For this review, take the finished solid that the model builds, in its own axes (mm). Face numbers are marked on the shaded views. A direction names the side the tool comes from. Round coordinates to 2 decimals unless told otherwise and drop trailing zeros. Write each loop counter-clockwise with the first axis right and the second up, starting at its lowest first coordinate (ties: lowest second). Pieces come first, ordered by that corner, then holes. Notation, with made-up numbers: M -5.5,52.5 L 43.5,52.5 A11 ccw 43.5,68.5 Z; hole C -13.5,33.25 d10. An arc over 180 degrees is marked long. Answer in a Markdown table with one row per item.
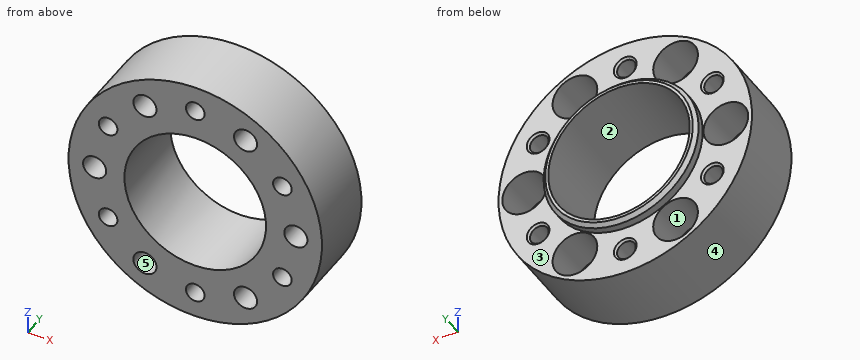
```python
from build123d import *

# Parameters (mm, degrees)
SKETCH_1_R                   = 17
SKETCH_1_R_2                 = 1.55
SKETCH_1_R_3                 = 9.5
EXTRUDE_1_DEPTH              = 9.5
HOLE_WIZARD_M3_1_D           = 2.5
HOLE_WIZARD_M3_1_CSINK_D     = 3.05
HOLE_WIZARD_M3_1_CSINK_ANGLE = 90
SKETCH_7_R                   = 10.4
SKETCH_7_R_2                 = 9.5
EXTRUDE_2_DEPTH              = 1.5
SKETCH_5_R                   = 3
CUT_EXTRUDE_1_DEPTH          = 5.5
CHAMFER_1_SIZE               = 0.5


with BuildPart() as part:
    # 草图1 → 凸台-拉伸1 (new body)
    with BuildSketch(Plane(origin=(0, 0, 0), x_dir=(1, 0, 0), z_dir=(0, 1, 0))):
        with Locations(Location((0, 0, 0), (0, 0, 270))):
            Circle(SKETCH_1_R)
        with Locations(Location((13.5, 0, 0), (0, 0, 270))):
            Circle(SKETCH_1_R_2, mode=Mode.SUBTRACT)
        with Locations(Location((6.75, -11.691342951, 0), (0, 0, 270))):
            Circle(SKETCH_1_R_2, mode=Mode.SUBTRACT)
        with Locations(Location((-6.75, -11.691342951, 0), (0, 0, 270))):
            Circle(SKETCH_1_R_2, mode=Mode.SUBTRACT)
        with Locations(Location((-13.5, 0, 0), (0, 0, 270))):
            Circle(SKETCH_1_R_2, mode=Mode.SUBTRACT)
        with Locations(Location((-6.75, 11.691342951, 0), (0, 0, 270))):
            Circle(SKETCH_1_R_2, mode=Mode.SUBTRACT)
        with Locations(Location((6.75, 11.691342951, 0), (0, 0, 270))):
            Circle(SKETCH_1_R_2, mode=Mode.SUBTRACT)
        with Locations(Location((0, 0, 0), (0, 0, 270))):
            Circle(SKETCH_1_R_3, mode=Mode.SUBTRACT)
    extrude(amount=EXTRUDE_1_DEPTH)

    # M3 螺纹孔1 (through all)
    with Locations(Plane(origin=(0, 9.5, 0), x_dir=(1, 0, 0), z_dir=(0, 1, 0))):
        with Locations((11.691342951, 6.75), (11.691342951, -6.75), (0, -13.5), (-11.691342951, -6.75), (-11.691342951, 6.75), (0, 13.5), (0, 0)):
            CounterSinkHole(HOLE_WIZARD_M3_1_D / 2, HOLE_WIZARD_M3_1_CSINK_D / 2, counter_sink_angle=HOLE_WIZARD_M3_1_CSINK_ANGLE)

    # 草图7 → 凸台-拉伸2 (add)
    with BuildSketch(Plane(origin=(0, 9.5, 0), x_dir=(1, 0, 0), z_dir=(0, 1, 0))):
        with Locations(Location((0, 0, 0), (0, 0, 270))):
            Circle(SKETCH_7_R)
        with Locations(Location((0, 0, 0), (0, 0, 270))):
            Circle(SKETCH_7_R_2, mode=Mode.SUBTRACT)
    extrude(amount=EXTRUDE_2_DEPTH)

    # 草图5 → 切除-拉伸1 (cut)
    with BuildSketch(Plane(origin=(0, 9.5, 0), x_dir=(1, 0, 0), z_dir=(0, 1, 0))):
        with Locations(Location((13.5, 0, 0), (0, 0, 270))):
            Circle(SKETCH_5_R)
        with Locations(Location((6.75, -11.691342951, 0), (0, 0, 270))):
            Circle(SKETCH_5_R)
        with Locations(Location((-6.75, -11.691342951, 0), (0, 0, 270))):
            Circle(SKETCH_5_R)
        with Locations(Location((-13.5, 0, 0), (0, 0, 270))):
            Circle(SKETCH_5_R)
        with Locations(Location((-6.75, 11.691342951, 0), (0, 0, 270))):
            Circle(SKETCH_5_R)
        with Locations(Location((6.75, 11.691342951, 0), (0, 0, 270))):
            Circle(SKETCH_5_R)
    extrude(amount=-CUT_EXTRUDE_1_DEPTH, mode=Mode.SUBTRACT)

    # 倒角1
    chamfer_1_edges = [part.edges().sort_by_distance(p)[0] for p in [
        (0, 11, -10.4),
    ]]
    chamfer(chamfer_1_edges, length=CHAMFER_1_SIZE)


solid = part.part
```
Q1. Machinability: for the marked faces 1 and 2, which of the approach directions +Z, -Z, +X, -X, +Y, -Y give a long, thin tool a straight path to every point of the face, cutting with its end or side? Answer none if there is none.
Found:
| item | result |
|---|---|
| face 1 | +Y |
| face 2 | +Y, -Y |
Q2. Take a section at B-B (x = -14.5). State the section outline as (y, z) points, then the cut area to 3 significant figures.
Found:
| item | result |
|---|---|
| outline | M 0,-8.87 L 9.5,-8.87 L 9.5,-2.83 L 4,-2.83 L 4,-1.18 L 0,-1.18 Z; M 0,1.18 L 4,1.18 L 4,2.83 L 9.5,2.83 L 9.5,8.87 L 0,8.87 Z |
| area | 128 mm² |
Q3. Mouldability with a two-part tool opening along X and no side actions: class the marked faces 3, 4 and 5 as +X half, -X half, draft (parallel to the pull), parting line (faces both ways), or undercut.
Found:
| item | result |
|---|---|
| face 3 | draft |
| face 4 | parting line |
| face 5 | undercut |
Q4. Insertion check: P1, Ø3, axis at x = -5.5, z = 11.5, coming from the +Y side; P2, Ø10, axis at x = 13, z = -5.5, coming from the -Y side; P3, Ø6, axis at x = -13, z = 1.5, coming from the +Y side; P4, Ø2, axis at x = 11.5, y = 1.5, coming from the -Z side. Each pin has a flat end and moves straight along its axis. Give the tip position at first contact, or say it passes through.
Found:
| item | result |
|---|---|
| P1 | y = 4 |
| P2 | y = 0 |
| P3 | y = 10.81 |
| P4 | z = -13.37 |
Q5. Take a section at A-A (y = 0.75). State how many separate pieces and enclosed holes the cut face has, then the cut area to 3 significant figures.
Found:
| item | result |
|---|---|
| separate pieces | 1 |
| enclosed holes | 13 |
| area | 550 mm² |
Q6. For probe 1 along X at (y, z) = (8.05, 0); probe 2 along Z at (x, y) = (-4, 9); probe 3 along Z at (x, y) = (-7, 5.5), list the stretches that pass through material, from the lowest coordinate up.
Found:
| item | result |
|---|---|
| probe 1 | -17 to -16.5, -10.5 to -9.5, 9.5 to 10.5, 16.5 to 17 |
| probe 2 | -16.52 to -12.89, -10.49 to -8.62, 8.62 to 10.49, 12.89 to 16.52 |
| probe 3 | -15.49 to -14.68, -8.7 to -6.42, 6.42 to 8.7, 14.68 to 15.49 |
